from build123d import *

# Parameters (mm, degrees)
THREE_ARM_BODY_50MM_DEPTH = 25
ARM_END_ROUND_B_RADIUS    = 25
ARM_END_ROUND_B_LENGTH    = 10.207259422
ARM_EDGE_FILLET_1_RADIUS  = 25
ARM_EDGE_FILLET_1_LENGTH  = 10.207259422
ARM_END_ROUND_A_RADIUS    = 25
ARM_END_ROUND_A_LENGTH    = 10.207259422
ARM_EDGE_FILLET_2_RADIUS  = 25
ARM_EDGE_FILLET_2_LENGTH  = 10.207259422
ARM_EDGE_FILLET_3_RADIUS  = 25
ARM_EDGE_FILLET_3_LENGTH  = 10.207259422
ARM_END_ROUND_C_RADIUS    = 25
ARM_END_ROUND_C_LENGTH    = 10.207259422
PIN_HOLE_A_15_REACH       = 188.921
PIN_HOLE_A_SKETCH_R       = 7.5
PIN_HOLE_B_15_REACH       = 188.921
PIN_HOLE_B_SKETCH_R       = 7.5
PIN_HOLE_C_15_REACH       = 183.779
PIN_HOLE_C_SKETCH_R       = 7.5
CENTER_BORE_SKETCH_R      = 10
CENTER_BORE_20_DEPTH      = 50
HUB_FILLET_R5_1_R         = 5
HUB_FILLET_R5_2_R         = 5
BORE_CHAMFER_1X45_SIZE    = 1


with BuildPart() as part:
    # Three-Arm Profile Sketch → Three-Arm Body 50mm (new, symmetric)
    with BuildSketch(Plane(origin=(0, 0, 0), x_dir=(1, 0, 0), z_dir=(0, 1, 0))):
        Polygon((-20.207259422, 35), (-20.207259422, 120), (-10, 120), (-10, 35), (10, 35), (10, 120), (20.207259422, 120), (20.207259422, 35), (40.414518843, 0), (114.026678165, -42.5), (108.923048454, -51.339745962), (35.310889132, -8.839745962), (25.310889132, -26.160254038), (98.923048454, -68.660254038), (93.819418743, -77.5), (20.207259422, -35), (-20.207259422, -35), (-93.819418743, -77.5), (-98.923048454, -68.660254038), (-25.310889132, -26.160254038), (-35.310889132, -8.839745962), (-108.923048454, -51.339745962), (-114.026678165, -42.5), (-40.414518843, 0), align=None)
    extrude(amount=THREE_ARM_BODY_50MM_DEPTH, both=True)

    # Arm End Round B: full round fillet: the end face becomes a half cylinder, R = half its width
    arm_end_round_b_face = Plane((-96.371233599, 0, 73.080127019), x_dir=(0.5, 0, 0.866025403784), z_dir=(-0.866025403784, 0, 0.5))  # on the end face: x along it, z out of the body
    arm_end_round_b_slab = arm_end_round_b_face.offset(-ARM_END_ROUND_B_RADIUS / 2) * Box(ARM_END_ROUND_B_LENGTH, 2 * ARM_END_ROUND_B_RADIUS, ARM_END_ROUND_B_RADIUS, mode=Mode.PRIVATE)  # the body's end, R deep
    arm_end_round_b_round = Plane((-74.720598504, 0, 60.580127019), x_dir=(-0.866025403784, 0, 0.5), z_dir=(0.5, 0, 0.866025403784)) * Cylinder(ARM_END_ROUND_B_RADIUS, ARM_END_ROUND_B_LENGTH, mode=Mode.PRIVATE)  # its axis R under the face
    add(arm_end_round_b_slab - arm_end_round_b_round, mode=Mode.SUBTRACT)

    # Arm Edge Fillet 1: full round fillet: the end face becomes a half cylinder, R = half its width
    arm_edge_fillet_1_face = Plane((-111.47486331, 0, 46.919872981), x_dir=(0.5, 0, 0.866025403784), z_dir=(-0.866025403784, 0, 0.5))  # on the end face: x along it, z out of the body
    arm_edge_fillet_1_slab = arm_edge_fillet_1_face.offset(-ARM_EDGE_FILLET_1_RADIUS / 2) * Box(ARM_EDGE_FILLET_1_LENGTH, 2 * ARM_EDGE_FILLET_1_RADIUS, ARM_EDGE_FILLET_1_RADIUS, mode=Mode.PRIVATE)  # the body's end, R deep
    arm_edge_fillet_1_round = Plane((-89.824228215, 0, 34.419872981), x_dir=(-0.866025403784, 0, 0.5), z_dir=(0.5, 0, 0.866025403784)) * Cylinder(ARM_EDGE_FILLET_1_RADIUS, ARM_EDGE_FILLET_1_LENGTH, mode=Mode.PRIVATE)  # its axis R under the face
    add(arm_edge_fillet_1_slab - arm_edge_fillet_1_round, mode=Mode.SUBTRACT)

    # Arm End Round A: full round fillet: the end face becomes a half cylinder, R = half its width
    arm_end_round_a_face = Plane((96.371233599, 0, 73.080127019), x_dir=(0.5, 0, -0.866025403784), z_dir=(0.866025403784, 0, 0.5))  # on the end face: x along it, z out of the body
    arm_end_round_a_slab = arm_end_round_a_face.offset(-ARM_END_ROUND_A_RADIUS / 2) * Box(ARM_END_ROUND_A_LENGTH, 2 * ARM_END_ROUND_A_RADIUS, ARM_END_ROUND_A_RADIUS, mode=Mode.PRIVATE)  # the body's end, R deep
    arm_end_round_a_round = Plane((74.720598504, 0, 60.580127019), x_dir=(0.866025403784, 0, 0.5), z_dir=(0.5, 0, -0.866025403784)) * Cylinder(ARM_END_ROUND_A_RADIUS, ARM_END_ROUND_A_LENGTH, mode=Mode.PRIVATE)  # its axis R under the face
    add(arm_end_round_a_slab - arm_end_round_a_round, mode=Mode.SUBTRACT)

    # Arm Edge Fillet 2: full round fillet: the end face becomes a half cylinder, R = half its width
    arm_edge_fillet_2_face = Plane((111.47486331, 0, 46.919872981), x_dir=(0.5, 0, -0.866025403784), z_dir=(0.866025403784, 0, 0.5))  # on the end face: x along it, z out of the body
    arm_edge_fillet_2_slab = arm_edge_fillet_2_face.offset(-ARM_EDGE_FILLET_2_RADIUS / 2) * Box(ARM_EDGE_FILLET_2_LENGTH, 2 * ARM_EDGE_FILLET_2_RADIUS, ARM_EDGE_FILLET_2_RADIUS, mode=Mode.PRIVATE)  # the body's end, R deep
    arm_edge_fillet_2_round = Plane((89.824228215, 0, 34.419872981), x_dir=(0.866025403784, 0, 0.5), z_dir=(0.5, 0, -0.866025403784)) * Cylinder(ARM_EDGE_FILLET_2_RADIUS, ARM_EDGE_FILLET_2_LENGTH, mode=Mode.PRIVATE)  # its axis R under the face
    add(arm_edge_fillet_2_slab - arm_edge_fillet_2_round, mode=Mode.SUBTRACT)

    # Arm Edge Fillet 3: full round fillet: the end face becomes a half cylinder, R = half its width
    arm_edge_fillet_3_face = Plane((15.103629711, 0, -120), x_dir=(-1, 0, 0), z_dir=(0, 0, -1))  # on the end face: x along it, z out of the body
    arm_edge_fillet_3_slab = arm_edge_fillet_3_face.offset(-ARM_EDGE_FILLET_3_RADIUS / 2) * Box(ARM_EDGE_FILLET_3_LENGTH, 2 * ARM_EDGE_FILLET_3_RADIUS, ARM_EDGE_FILLET_3_RADIUS, mode=Mode.PRIVATE)  # the body's end, R deep
    arm_edge_fillet_3_round = Plane((15.103629711, 0, -95), x_dir=(0, 0, -1), z_dir=(-1, 0, 0)) * Cylinder(ARM_EDGE_FILLET_3_RADIUS, ARM_EDGE_FILLET_3_LENGTH, mode=Mode.PRIVATE)  # its axis R under the face
    add(arm_edge_fillet_3_slab - arm_edge_fillet_3_round, mode=Mode.SUBTRACT)

    # Arm End Round C: full round fillet: the end face becomes a half cylinder, R = half its width
    arm_end_round_c_face = Plane((-15.103629711, 0, -120), x_dir=(1, 0, 0), z_dir=(0, 0, -1))  # on the end face: x along it, z out of the body
    arm_end_round_c_slab = arm_end_round_c_face.offset(-ARM_END_ROUND_C_RADIUS / 2) * Box(ARM_END_ROUND_C_LENGTH, 2 * ARM_END_ROUND_C_RADIUS, ARM_END_ROUND_C_RADIUS, mode=Mode.PRIVATE)  # the body's end, R deep
    arm_end_round_c_round = Plane((-15.103629711, 0, -95), x_dir=(0, 0, -1), z_dir=(1, 0, 0)) * Cylinder(ARM_END_ROUND_C_RADIUS, ARM_END_ROUND_C_LENGTH, mode=Mode.PRIVATE)  # its axis R under the face
    add(arm_end_round_c_slab - arm_end_round_c_round, mode=Mode.SUBTRACT)

    # Pin Hole A _15: up to this face of the body (flat: up to its plane)
    pin_hole_a_15_end = Plane(part.part.faces().sort_by_distance((75.066762447, 0, 20.006482173))[0])
    # Pin Hole A Sketch → Pin Hole A _15 (cut, up to the picked face)
    with BuildSketch(Plane(origin=(-10.103629711, 0, 17.5), x_dir=(0.8660254037844392, 0, 0.49999999999999917), z_dir=(-0.49999999999999917, 0, 0.8660254037844392)), mode=Mode.PRIVATE) as pin_hole_a_15_sk1:
        with Locations((95, 0)):
            Circle(PIN_HOLE_A_SKETCH_R)
    pin_hole_a_15_tool1 = split(extrude(pin_hole_a_15_sk1.sketch, amount=-PIN_HOLE_A_15_REACH, mode=Mode.PRIVATE), bisect_by=pin_hole_a_15_end, keep=Keep.BOTH, mode=Mode.PRIVATE)
    add(pin_hole_a_15_tool1.solids().sort_by(Axis((72.168784, 0, 65), (0.49999999999999917, 0, -0.8660254037844392)))[0], mode=Mode.SUBTRACT)

    # Pin Hole B _15: up to this face of the body (flat: up to its plane)
    pin_hole_b_15_end = Plane(part.part.faces().sort_by_distance((-75.066762447, 0, 20.006482173))[0])
    # Pin Hole B Sketch → Pin Hole B _15 (cut, up to the picked face)
    with BuildSketch(Plane(origin=(10.103629711, 0, 17.5), x_dir=(0.86602540378444, 0, -0.4999999999999976), z_dir=(0.4999999999999976, 0, 0.86602540378444)), mode=Mode.PRIVATE) as pin_hole_b_15_sk1:
        with Locations((-95, 0)):
            Circle(PIN_HOLE_B_SKETCH_R)
    pin_hole_b_15_tool1 = split(extrude(pin_hole_b_15_sk1.sketch, amount=-PIN_HOLE_B_15_REACH, mode=Mode.PRIVATE), bisect_by=pin_hole_b_15_end, keep=Keep.BOTH, mode=Mode.PRIVATE)
    add(pin_hole_b_15_tool1.solids().sort_by(Axis((-72.168784, 0, 65), (-0.4999999999999976, 0, -0.86602540378444)))[0], mode=Mode.SUBTRACT)

    # Pin Hole C _15: up to this face of the body (flat: up to its plane)
    pin_hole_c_15_end = Plane(part.part.faces().sort_by_distance((20.207259422, 0, -75.012964345))[0])
    # Pin Hole C Sketch → Pin Hole C _15 (cut, up to the picked face)
    with BuildSketch(Plane.ZY.offset(20.207259422), mode=Mode.PRIVATE) as pin_hole_c_15_sk1:
        with Locations((-95, 0)):
            Circle(PIN_HOLE_C_SKETCH_R)
    pin_hole_c_15_tool1 = split(extrude(pin_hole_c_15_sk1.sketch, amount=-PIN_HOLE_C_15_REACH, mode=Mode.PRIVATE), bisect_by=pin_hole_c_15_end, keep=Keep.BOTH, mode=Mode.PRIVATE)
    add(pin_hole_c_15_tool1.solids().sort_by(Axis((-20.207259, 0, -95), (1, 0, 0)))[0], mode=Mode.SUBTRACT)

    # Center Bore Sketch → Center Bore _20 (cut)
    with BuildSketch(Plane.XZ.offset(25)):
        with Locations(Location((0, 0, 0), (0, 0, 270))):
            Circle(CENTER_BORE_SKETCH_R)
    extrude(amount=-CENTER_BORE_20_DEPTH, mode=Mode.SUBTRACT)

    # Hub Fillet R5 1
    hub_fillet_r5_1_edges = [part.edges().sort_by_distance(p)[0] for p in [
        (35.310889132, 0, 8.839745962),
        (25.310889132, 0, 26.160254038),
        (-25.310889132, 0, 26.160254038),
        (-35.310889132, 0, 8.839745962),
        (-10, 0, -35),
        (10, 0, -35),
    ]]
    fillet(hub_fillet_r5_1_edges, radius=HUB_FILLET_R5_1_R)

    # Hub Fillet R5 2
    hub_fillet_r5_2_edges = [part.edges().sort_by_distance(p)[0] for p in [
        (20.207259422, 0, -35),
        (40.414518843, 0, 0),
        (20.207259422, 0, 35),
        (-20.207259422, 0, 35),
        (-40.414518843, 0, 0),
        (-20.207259422, 0, -35),
    ]]
    fillet(hub_fillet_r5_2_edges, radius=HUB_FILLET_R5_2_R)

    # Bore Chamfer 1x45
    bore_chamfer_1x45_edges = [part.edges().sort_by_distance(p)[0] for p in [
        (0, -25, 10),
        (0, 25, 10),
    ]]
    chamfer(bore_chamfer_1x45_edges, length=BORE_CHAMFER_1X45_SIZE)


solid = part.part
Read the model definition and answer for the solid it produces. Units are mm, in the model's axes. A direction names the side the tool comes from. Round coordinates to 2 decimals unless told otherwise and drop trailing zeros. Loops run counter-clockwise (first coordinate to the right, second up) from the corner with the lowest first, then second, coordinate; pieces in that order, holes last.
Q1. Which of the six approach directions +Z, -Z, +X, -X, +Y, -Y give full straight-line access (tool end or side, diameter ignored) to faces 5 (the face through (-20.207, 0, -78)), 6 (the face through (58.101, 0.35, 56.878)), 7 (the face through (10, 0, -79))?
Q2. Determine the mould class of faces 1 (the face through (0, 0, 35)), 2 (the face through (-10, 0, -81)), 3 (the face through (-73.8, 0.35, 31.06)), 4 (the face through (-35.794, -0.35, 10.855)) for opening direction Z: released by +Z, released by -Z, zero draft, split by the parting line, or undercut.
Q3. Section D-D on x = -57 is taken. Write down the section's boundary in (y, z), and give its area (3 significant figures).
Q4. Consider probe 1 along Y at (x, z) = (17.5, -95); probe 2 along X at (y, z) = (-9.5, -93.5); probe 3 along X at (y, z) = (-13, 69). Determine where each line is inside the solid, lowest interval first.
Q5. Section A-A on z = -66.5 is taken. Write down the section's boundary in (x, y), and give its area (3 significant figures).
Q6. Section C-C on y = 0 is taken. Give the number of separate pieces and of enclosed holes in the cut face, and give its area (3 significant figures).
Q7. Each of these flat-tipped pins is pushed along its axis until it touches: pin 1 (12 mm diameter, centred on y = -14.5, z = 25, fed in from +X); pin 2 (3 mm diameter, centred on x = 80.5, y = 6.5, fed in from +Z); pin 3 (15 mm diameter, centred on y = -2.5, z = -66.5, fed in from +X); pin 4 (12 mm diameter, centred on x = 0, z = 0, fed in from +Y). Where does it stop, or does it pass through?
Q8. Section B-B on x = 0 is taken. Write down the section's boundary in (y, z), and give its area (3 significant figures).
Output:
1. face 5: -Z, -X, +Y, -Y
1. face 6: +Z, +Y, -Y
1. face 7: -Z, +Y, -Y
2. face 1: released by +Z
2. face 2: zero draft
2. face 3: undercut
2. face 4: undercut
3. outline: (-25, 9.58) - (25, 9.58) - (25, 21.36) - (-25, 21.36) - close; (-25, 44.46) - (25, 44.46) - (25, 56.24) - (-25, 56.24) - close
3. area: 1,180 mm2
4. probe 1: y = -25 to -7.5, 7.5 to 25
4. probe 2: x = -20.21 to -10, 10 to 20.21
4. probe 3: x = -94.52 to -79.1, 79.1 to 94.52
5. outline: (-20.21, -25) - (-10, -25) - (-10, 25) - (-20.21, 25) - close; (10, -25) - (20.21, -25) - (20.21, 25) - (10, 25) - close
5. area: 1,020 mm2
6. separate pieces: 7
6. enclosed holes: 1
6. area: 8,250 mm2
7. pin 1: stops at x = 94.11
7. pin 2: stops at z = 70.68
7. pin 3: stops at x = 20.21
7. pin 4: passes through
8. outline: (-25, -35) - (25, -35) - (25, -11) - (24, -10) - (-24, -10) - (-25, -11) - close; (-25, 11) - (-24, 10) - (24, 10) - (25, 11) - (25, 35) - (-25, 35) - close
8. area: 2,500 mm2
